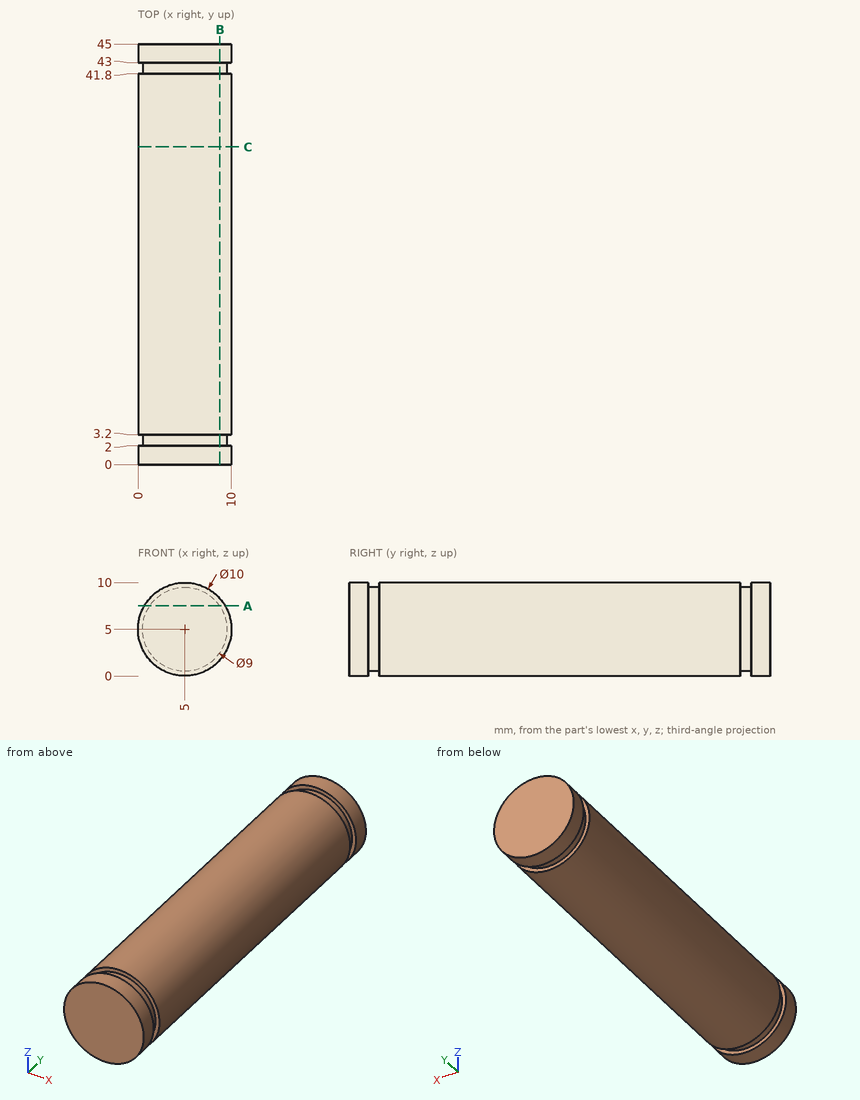
Input: dimensioned drawing with shaded views. Units: mm. Origin: part minimum x, y, z. Round coordinates to 2 decimals unless told otherwise and drop trailing zeros. Loops run counter-clockwise (first coordinate to the right, second up) from the corner with the lowest first, then second, coordinate; pieces in that order, holes last. Notation, with made-up numbers: M 88,8 L 115,8 A27 cw 115,28 Z; hole C 23,58.5 d2. An arc over 180 degrees is marked long. Return JSON: item names as keys, results as strings. Group by question number.
1. Material intervals for line 1 along Y through (x, z) = (8.25, 1.75); line 2 along X through (y, z) = (29, 4.75); line 3 along Z through (x, y) = (6.25, 6), sorted ascending. Write a range as from..to.
2. Pin query (flat end, axial travel): pin 1 (2 mm diameter, centred on y = 22.5, z = 9, fed in from -X). Return the tip coordinate at first contact, or that it passes through.
3. Section query A-A on z = 7.5. Output: boundary loops of the cut face in (x, y).
4. Section query B-B on x = 8.75. Output: boundary loops of the cut face in (y, z).
5. Section query C-C on y = 34. Output: boundary loops of the cut face in (x, z), and give its area (3 significant figures).
Checks:
{
 "1": {"line 1": "y = 0..2, 3.2..41.8, 43..45", "line 2": "x = 0.01..9.99", "line 3": "z = 0.16..9.84"},
 "2": {"pin 1": "stops at x = 1"},
 "3": {"outline": "M 0.67,0 L 9.33,0 L 9.33,2 L 8.74,2 L 8.74,3.2 L 9.33,3.2 L 9.33,41.8 L 8.74,41.8 L 8.74,43 L 9.33,43 L 9.33,45 L 0.67,45 L 0.67,43 L 1.26,43 L 1.26,41.8 L 0.67,41.8 L 0.67,3.2 L 1.26,3.2 L 1.26,2 L 0.67,2 Z"},
 "4": {"outline": "M 0,1.69 L 2,1.69 L 2,2.51 L 3.2,2.51 L 3.2,1.69 L 41.8,1.69 L 41.8,2.51 L 43,2.51 L 43,1.69 L 45,1.69 L 45,8.31 L 43,8.31 L 43,7.49 L 41.8,7.49 L 41.8,8.31 L 3.2,8.31 L 3.2,7.49 L 2,7.49 L 2,8.31 L 0,8.31 Z"},
 "5": {"outline": "C 5,5 d10", "area": "78.5 mm²"}
}
